Verification items for the finished model (mm, model axes). A direction names the side the tool comes from. Give positions to 0.01 mm unless a question says otherwise; leave off trailing zeros. Loops run counter-clockwise (first coordinate to the right, second up) from the corner with the lowest first, then second, coordinate; pieces in that order, holes last. Notation, with made-up numbers: (-2.5, 3.5) - (27.5, 3.5) arc R31 ccw to (27.5, 39.5) - close; hole circle Ø1 at (69, 51). An arc over 180 degrees is marked (long way). One line per item, written item: value. Start each with the question number.
1. Sectioned sample at C-C (y = 37.5). Record the cut outline in (x, z).
2. Sectioned sample at B-B (x = 9.5). Record the cut outline in (y, z).
3. Sectioned sample at D-D (z = 2.45). Count the separate pieces of the cut face and the enclosed holes in it, plus the area to 3 significant figures.
4. Mould release check, pull along Y, two halves, no side actions. Record for faces 3 (the flat face through (-1, 1, 3)), 4 (the flat face through (33, 16, 1)), 5 (the cylindrical face through (2.439, 5.018, 1.479)): pulls with the +Y half, pulls with the -Y half, needs draft (parallel to the pull), parting line crosses it, or undercut.
5. Access from +Z, -Z, +X, -X, +Y, -Y to the whole of each face (thin tool, end or side, straight path). Record for faces 1 (the flat face through (-33, 16, 1)), 2 (the flat face through (-37.5, 0, 1)).
6. Scan lines: L1, parallel to Y at x = 0, z = 2.4; L2, parallel to X at y = 14.5, z = 2.6; L3, parallel to X at y = 16.5, z = 0.4. Record each from-to range of solid material in increasing order. Write a range as [from, to].
7. Sectioned sample at A-A (y = -5.5). Record the cut outline in (x, z).
8. Gauge pin test, flat ends, axial feed: pin 1 (3 mm diameter, centred on x = 15.2, y = 31.2, fed in from +Z); pin 2 (1.5 mm diameter, centred on x = -3, z = 1, fed in from +Y); pin 3 (1 mm diameter, centred on x = 6, z = 1, fed in from +Y); pin 4 (0.9 mm diameter, centred on x = 32.5, z = 1, fed in from +Y). Record the tip position at first contact, or that the pin passes through.
from build123d import *

# Parameters (mm, degrees)
SKETCH_1_W                  = 75
SKETCH_1_H                  = 32
EXTRUDE_1_DEPTH             = 3
SKETCH_2_R                  = 26
EXTRUDE_3_DEPTH             = 3
FILLET_1_R                  = 3
SKETCH_3_R                  = 11.25
CUT_EXTRUDE_1_DEPTH         = 57.384838388
HOLE_WIZARD_M3_1_AT_2_COUNT = 2
HOLE_WIZARD_M3_1_AT_2_PITCH = 16.455387592
HOLE_WIZARD_M3_1_AT_3_COUNT = 2
HOLE_WIZARD_M3_1_AT_3_PITCH = 30.405591591
HOLE_WIZARD_M3_1_AT_4_COUNT = 2
HOLE_WIZARD_M3_1_AT_4_PITCH = 39.726819898
HOLE_WIZARD_M3_1_AT_5_COUNT = 2
HOLE_WIZARD_M3_1_AT_5_PITCH = 43
HOLE_WIZARD_M3_1_AT_6_COUNT = 2
HOLE_WIZARD_M3_1_AT_6_PITCH = 39.726819898
HOLE_WIZARD_M3_1_AT_7_COUNT = 2
HOLE_WIZARD_M3_1_AT_7_PITCH = 30.405591591
HOLE_WIZARD_M3_1_AT_8_COUNT = 2
HOLE_WIZARD_M3_1_AT_8_PITCH = 16.455387592


with BuildPart() as part:
    # 草图1 → 凸台-拉伸1 (new body)
    with BuildSketch(Plane.XY):
        Rectangle(SKETCH_1_W, SKETCH_1_H)
    extrude(amount=EXTRUDE_1_DEPTH)

    # 草图2 → 凸台-拉伸3 (add, through all)
    with BuildSketch(Plane.XY.offset(3)):
        with Locations((0, 16)):
            Circle(SKETCH_2_R)
    extrude(amount=-EXTRUDE_3_DEPTH)

    # 圆角1
    fillet_1_edges = [part.edges().sort_by_distance(p)[0] for p in [
        (26, 16, 1.5),
        (-26, 16, 1.5),
    ]]
    fillet(fillet_1_edges, radius=FILLET_1_R)

    # 草图3 → 切除-拉伸1 (cut, through all)
    with BuildSketch(Plane(origin=(0, 0, 0), x_dir=(-1, 0, 0), z_dir=(0, 0, -1))):
        with Locations((0, 16)):
            Circle(SKETCH_3_R)
    extrude(amount=-CUT_EXTRUDE_1_DEPTH, mode=Mode.SUBTRACT)

    # 草图5 → M3 六角凹锥坑螺钉的锥形沉头孔1 (revolve, cut)
    with BuildSketch(Plane(origin=(0, 37.5, 0), x_dir=(0, 1, 0), z_dir=(1, 0, 0))):
        Polygon((0, 0), (0, 3), (1.7, 3), (1.7, 1.66), (3.36, 0), align=None)
    hole_wizard_m3_1 = revolve(axis=Axis((0, 37.5, -6.35), (0, 0, 1)), mode=Mode.SUBTRACT)

    # M3 六角凹锥坑螺钉的锥形沉头孔1 at 2: M3 六角凹锥坑螺钉的锥形沉头孔1 ×2
    with Locations(*[Vector(-0.9238795325112867, -0.38268343236508967, 0) * (i * HOLE_WIZARD_M3_1_AT_2_PITCH) for i in range(1, HOLE_WIZARD_M3_1_AT_2_COUNT)]):
        add(hole_wizard_m3_1, mode=Mode.SUBTRACT)

    # M3 六角凹锥坑螺钉的锥形沉头孔1 at 3: M3 六角凹锥坑螺钉的锥形沉头孔1 ×2
    with Locations(*[Vector(-0.7071067811865476, -0.7071067811865475, 0) * (i * HOLE_WIZARD_M3_1_AT_3_PITCH) for i in range(1, HOLE_WIZARD_M3_1_AT_3_COUNT)]):
        add(hole_wizard_m3_1, mode=Mode.SUBTRACT)

    # M3 六角凹锥坑螺钉的锥形沉头孔1 at 4: M3 六角凹锥坑螺钉的锥形沉头孔1 ×2
    with Locations(*[Vector(-0.38268343236508995, -0.9238795325112867, 0) * (i * HOLE_WIZARD_M3_1_AT_4_PITCH) for i in range(1, HOLE_WIZARD_M3_1_AT_4_COUNT)]):
        add(hole_wizard_m3_1, mode=Mode.SUBTRACT)

    # M3 六角凹锥坑螺钉的锥形沉头孔1 at 5: M3 六角凹锥坑螺钉的锥形沉头孔1 ×2
    with Locations(*[(0, -i * HOLE_WIZARD_M3_1_AT_5_PITCH, 0) for i in range(1, HOLE_WIZARD_M3_1_AT_5_COUNT)]):
        add(hole_wizard_m3_1, mode=Mode.SUBTRACT)

    # M3 六角凹锥坑螺钉的锥形沉头孔1 at 6: M3 六角凹锥坑螺钉的锥形沉头孔1 ×2
    with Locations(*[Vector(0.38268343236508967, -0.9238795325112868, 0) * (i * HOLE_WIZARD_M3_1_AT_6_PITCH) for i in range(1, HOLE_WIZARD_M3_1_AT_6_COUNT)]):
        add(hole_wizard_m3_1, mode=Mode.SUBTRACT)

    # M3 六角凹锥坑螺钉的锥形沉头孔1 at 7: M3 六角凹锥坑螺钉的锥形沉头孔1 ×2
    with Locations(*[Vector(0.7071067811865474, -0.7071067811865477, 0) * (i * HOLE_WIZARD_M3_1_AT_7_PITCH) for i in range(1, HOLE_WIZARD_M3_1_AT_7_COUNT)]):
        add(hole_wizard_m3_1, mode=Mode.SUBTRACT)

    # M3 六角凹锥坑螺钉的锥形沉头孔1 at 8: M3 六角凹锥坑螺钉的锥形沉头孔1 ×2
    with Locations(*[Vector(0.9238795325112868, -0.3826834323650898, 0) * (i * HOLE_WIZARD_M3_1_AT_8_PITCH) for i in range(1, HOLE_WIZARD_M3_1_AT_8_COUNT)]):
        add(hole_wizard_m3_1, mode=Mode.SUBTRACT)


solid = part.part
Results are:
1. outline: (-14.62, 0) - (-3.36, 0) - (-1.7, 1.66) - (-1.7, 3) - (-14.62, 3) - close; (1.7, 1.66) - (3.36, 0) - (14.62, 0) - (14.62, 3) - (1.7, 3) - close
2. outline: (-16, 0) - (9.97, 0) - (9.97, 3) - (-16, 3) - close; (22.03, 0) - (40.2, 0) - (40.2, 3) - (22.03, 3) - close
3. separate pieces: 1
3. enclosed holes: 9
3. area: 2,990 mm^2
4. face 3: needs draft
4. face 4: pulls with the +Y half
4. face 5: undercut
5. face 1: +Z, -Z, -X, +Y
5. face 2: +Z, -Z, -X, +Y, -Y
6. L1: y = [-16, -7.2], [-3.8, 4.75], [27.25, 35.8], [39.2, 42]
6. L2: x = [-37.5, -22.3], [-20.7, -11.15], [11.15, 20.7], [22.3, 37.5]
6. L3: x = [-27.19, -24.42], [-18.58, -11.24], [11.24, 18.58], [24.42, 27.19]
7. outline: (-37.5, 0) - (-3.36, 0) - (-1.7, 1.66) - (-1.7, 3) - (-37.5, 3) - close; (1.7, 1.66) - (3.36, 0) - (37.5, 0) - (37.5, 3) - (1.7, 3) - close
8. pin 1: passes through
8. pin 2: stops at y = 41.9
8. pin 3: stops at y = 41.41
8. pin 4: stops at y = 16
